from build123d import *

# Parameters (mm, degrees)
M4_TAPPED_HOLE1_D                       = 3.3
M4_TAPPED_HOLE1_DEPTH                   = 11.5
M4_TAPPED_HOLE1_TIP                     = 0.991420021
CUT_EXTRUDE2_REACH                      = 97
CBORE_FOR_M4_HEX_HEAD_BOLT1_D           = 3
CBORE_FOR_M4_HEX_HEAD_BOLT1_CBORE_D     = 8
CBORE_FOR_M4_HEX_HEAD_BOLT1_CBORE_DEPTH = 3
M4_TAPPED_HOLE4_D                       = 3.3
M4_TAPPED_HOLE4_DEPTH                   = 10.1
M4_TAPPED_HOLE4_TIP                     = 0.991420021
CBORE_FOR_M4_HEX_HEAD_BOLT2_D           = 4.5
CBORE_FOR_M4_HEX_HEAD_BOLT2_DEPTH       = 10.1
CBORE_FOR_M4_HEX_HEAD_BOLT2_CBORE_D     = 8
CBORE_FOR_M4_HEX_HEAD_BOLT2_CBORE_DEPTH = 5
CBORE_FOR_M4_HEX_HEAD_BOLT2_TIP         = 1.351936393


with BuildPart() as part:
    # Sketch1 → Revolve1 (revolve)
    with BuildSketch(Plane.XY, mode=Mode.PRIVATE) as revolve1_sk:
        Polygon((0, 85), (-30, 85), (-30, 77), (-12.5, 77), (-12.5, 0), (0, 0), align=None)
    revolve(revolve1_sk.sketch.rotate(Axis((0, 0, 0), (0, 1, 0)), 270), axis=Axis((0, 0, 0), (0, 1, 0)))

    # M4 Tapped Hole1
    with Locations(Plane(origin=(-8, 0, 0), x_dir=(0, 0, -1), z_dir=(0, -1, 0))):
        with Locations((0, 0), (0, 16)):
            Hole(M4_TAPPED_HOLE1_D / 2, depth=M4_TAPPED_HOLE1_DEPTH)
            with Locations((0, 0, -(M4_TAPPED_HOLE1_DEPTH + M4_TAPPED_HOLE1_TIP / 2))):  # 118° drill point
                Cone(0, M4_TAPPED_HOLE1_D / 2, M4_TAPPED_HOLE1_TIP, mode=Mode.SUBTRACT)

    # Sketch4 → Cut-Extrude2 (cut, up to next)
    with BuildSketch(Plane(origin=(0, 85, 0), x_dir=(1, 0, 0), z_dir=(0, 1, 0)), mode=Mode.PRIVATE) as cut_extrude2_sk1:
        with BuildLine():
            Line((22.360679775, 20), (-22.360679775, 20))
            ThreePointArc((-22.360679775, 20), (0, 30), (22.360679775, 20))
        make_face()
    cut_extrude2_tool1 = extrude(cut_extrude2_sk1.sketch, amount=-CUT_EXTRUDE2_REACH, mode=Mode.PRIVATE) & part.part
    # Sketch4 → Cut-Extrude2 (cut, up to next)
    with BuildSketch(Plane(origin=(0, 85, 0), x_dir=(1, 0, 0), z_dir=(0, 1, 0)), mode=Mode.PRIVATE) as cut_extrude2_sk2:
        with BuildLine():
            Line((22.360679775, -20), (-22.360679775, -20))
            ThreePointArc((-22.360679775, -20), (0, -30), (22.360679775, -20))
        make_face()
    cut_extrude2_tool2 = extrude(cut_extrude2_sk2.sketch, amount=-CUT_EXTRUDE2_REACH, mode=Mode.PRIVATE) & part.part
    add(cut_extrude2_tool1.solids().sort_by_distance((0, 85, -24.063287))[0], mode=Mode.SUBTRACT)
    add(cut_extrude2_tool2.solids().sort_by_distance((0, 85, 24.063287))[0], mode=Mode.SUBTRACT)

    # CBORE for M4 Hex Head Bolt1 (through all)
    with Locations(Plane(origin=(-20, 77, 0), x_dir=(0, 0, -1), z_dir=(0, -1, 0))):
        with Locations((0, 0), (0, 40)):
            CounterBoreHole(CBORE_FOR_M4_HEX_HEAD_BOLT1_D / 2, CBORE_FOR_M4_HEX_HEAD_BOLT1_CBORE_D / 2, CBORE_FOR_M4_HEX_HEAD_BOLT1_CBORE_DEPTH)

    # M4 Tapped Hole4
    with Locations(Plane(origin=(-20, 80, 0), x_dir=(0, 0, -1), z_dir=(0, -1, 0))):
        with Locations((0, 0), (0, 40)):
            Hole(M4_TAPPED_HOLE4_D / 2, depth=M4_TAPPED_HOLE4_DEPTH)
            with Locations((0, 0, -(M4_TAPPED_HOLE4_DEPTH + M4_TAPPED_HOLE4_TIP / 2))):  # 118° drill point
                Cone(0, M4_TAPPED_HOLE4_D / 2, M4_TAPPED_HOLE4_TIP, mode=Mode.SUBTRACT)

    # CBORE for M4 Hex Head Bolt2
    with Locations(Plane(origin=(-18, 77, 13), x_dir=(0, 0, -1), z_dir=(0, -1, 0))):
        with Locations((0, 0), (0, 36), (26, 36), (26, 0)):
            CounterBoreHole(CBORE_FOR_M4_HEX_HEAD_BOLT2_D / 2, CBORE_FOR_M4_HEX_HEAD_BOLT2_CBORE_D / 2, CBORE_FOR_M4_HEX_HEAD_BOLT2_CBORE_DEPTH, depth=CBORE_FOR_M4_HEX_HEAD_BOLT2_DEPTH)
            with Locations((0, 0, -(CBORE_FOR_M4_HEX_HEAD_BOLT2_DEPTH + CBORE_FOR_M4_HEX_HEAD_BOLT2_TIP / 2))):  # 118° drill point
                Cone(0, CBORE_FOR_M4_HEX_HEAD_BOLT2_D / 2, CBORE_FOR_M4_HEX_HEAD_BOLT2_TIP, mode=Mode.SUBTRACT)


solid = part.part
Part model, mm, in its own coordinate system. A direction names the side the tool comes from. Coordinates: 2 decimals unless noted, no trailing zeros. Order: outer loops, then holes, each group sorted by start corner. A loop starts at its lowest first (then second) coordinate and runs counter-clockwise, first axis right, second up. Notation, with made-up numbers: M 13.25,86 L 29.25,86 A21 ccw 29.25,90 Z; hole C 26.5,68 d2. An arc over 180 degrees is marked long. Use a Markdown table: item, result.
(1) Pull direction Z, two halves, no side cores. Call faces 1 (the flat face through (0, 81, -20)), 2 (the flat face through (13, 77, 0)), 3 (the cylindrical face through (30, 81, 0)), 4 (the cylindrical face through (9.115, 5.831, -1.216)): released by +Z, released by -Z, zero draft, split by the parting line, or undercut.
A:
| item | result |
|---|---|
| face 1 | released by -Z |
| face 2 | zero draft |
| face 3 | split by the parting line |
| face 4 | undercut |
(2) Cut at B-B on x = 0. Write the cut outline in (y, z).
A:
| item | result |
|---|---|
| outline | M 0,-12.5 L 77,-12.5 L 77,-20 L 85,-20 L 85,20 L 77,20 L 77,12.5 L 0,12.5 Z |
(3) Cut at C-C on y = 32. Write the cut outline in (x, z).
A:
| item | result |
|---|---|
| outline | C 0,0 d25 |
(4) Cut at D-D on z = 3. Write the cut outline in (x, y).
A:
| item | result |
|---|---|
| outline | M -29.85,77 L -22.65,77 L -22.65,80 L -17.35,80 L -17.35,77 L -12.13,77 L -12.13,0 L 12.13,0 L 12.13,77 L 17.35,77 L 17.35,80 L 22.65,80 L 22.65,77 L 29.85,77 L 29.85,85 L -29.85,85 Z |
(5) Tool access for faces 5 (the cylindrical face through (-15.3, 79.46, 15.95)), 6 (the cylindrical face through (-20.196, 83.521, -13.488)): list every direction of +Z, -Z, +X, -X, +Y, -Y with a clear straight run to the whole face (end or side of a thin tool).
A:
| item | result |
|---|---|
| face 5 | -Y |
| face 6 | +Y, -Y |
(6) Flat gauge pins, fed straight in: pin 1 (5 mm diameter, centred on x = -18, z = -13, fed in from -Y); pin 2 (12 mm diameter, centred on y = 21, z = 2.5, fed in from -X); pin 3 (10 mm diameter, centred on x = -20, z = -6.5, fed in from -Y). Where does each tip first touch, or does it go through?
A:
| item | result |
|---|---|
| pin 1 | stops at y = 82 |
| pin 2 | stops at x = -12.5 |
| pin 3 | stops at y = 77 |
(7) Probe L1, parallel to X at y = 81, z = 0; L2, parallel to X at y = 78, z = 0; L3, parallel to Y at x = 24.5, z = 10.5. List the from-to ranges inside material, lowest first.
A:
| item | result |
|---|---|
| L1 | x = -30 to -21.65, -18.35 to 18.35, 21.65 to 30 |
| L2 | x = -30 to -24, -16 to 16, 24 to 30 |
| L3 | y = 77 to 85 |
(8) Cut at A-A on x = 17. Write the cut outline in (y, z), then the cut area to 3 significant figures.
A:
| item | result |
|---|---|
| outline | M 77,-20 L 85,-20 L 85,-15.02 L 82,-15.02 L 82,-16.87 L 77,-16.87 Z; M 77,-9.13 L 82,-9.13 L 82,-10.98 L 85,-10.98 L 85,10.98 L 82,10.98 L 82,9.13 L 77,9.13 L 77,2.65 L 80,2.65 L 80,-2.65 L 77,-2.65 Z; M 77,16.87 L 82,16.87 L 82,15.02 L 85,15.02 L 85,20 L 77,20 Z |
| area | 202 mm^2 |
